For this review, take the finished solid that the model builds, in its own axes (mm). A direction names the side the tool comes from. Round coordinates to 2 decimals unless told otherwise and drop trailing zeros. Order: outer loops, then holes, each group sorted by start corner. A loop starts at its lowest first (then second) coordinate and runs counter-clockwise, first axis right, second up. Notation, with made-up numbers: M 5,33.25 L 9,33.25 A18 ccw 9,53.25 Z; hole C 11.25,60.25 d11. An arc over 180 degrees is marked long. Use a Markdown table: item, result.
from build123d import *

# Parameters (mm, degrees)
SKETCH1_W                              = 65
SKETCH1_H                              = 45
BOSS_EXTRUDE1_DEPTH                    = 45
SKETCH2_W                              = 15
SKETCH2_H                              = 10
CUT_EXTRUDE1_DEPTH                     = 40
SKETCH3_R                              = 5
BOSS_EXTRUDE2_DEPTH                    = 40
BOSS_EXTRUDE3_START                    = -40
BOSS_EXTRUDE3_DEPTH                    = 40
SKETCH5_R                              = 15
BOSS_EXTRUDE4_DEPTH                    = 2
CBORE_FOR_M2_HEX_CAP_SCREW2_AT_2_COUNT = 2
CBORE_FOR_M2_HEX_CAP_SCREW2_AT_2_PITCH = 50
CBORE_FOR_M2_HEX_CAP_SCREW2_AT_3_COUNT = 2
CBORE_FOR_M2_HEX_CAP_SCREW2_AT_3_PITCH = 35
CBORE_FOR_M2_HEX_CAP_SCREW2_AT_4_COUNT = 2
CBORE_FOR_M2_HEX_CAP_SCREW2_AT_4_PITCH = 61.032778079


with BuildPart() as part:
    # Sketch1 → Boss-Extrude1 (new body)
    with BuildSketch(Plane(origin=(0, 0, 0), x_dir=(1, 0, 0), z_dir=(0, 1, 0))):
        Rectangle(SKETCH1_W, SKETCH1_H)
    extrude(amount=BOSS_EXTRUDE1_DEPTH)

    # Sketch2 → Cut-Extrude1 (cut)
    with BuildSketch(Plane(origin=(0, 45, 0), x_dir=(1, 0, 0), z_dir=(0, 1, 0))):
        with Locations((-25, 17.5)):
            Rectangle(SKETCH2_W, SKETCH2_H)
        with Locations((-25, -17.5)):
            Rectangle(SKETCH2_W, SKETCH2_H)
        with Locations((25, -17.5)):
            Rectangle(SKETCH2_W, SKETCH2_H)
        with Locations((25, 17.5)):
            Rectangle(SKETCH2_W, SKETCH2_H)
    extrude(amount=-CUT_EXTRUDE1_DEPTH, mode=Mode.SUBTRACT)

    # Sketch3 → Boss-Extrude2 (add)
    with BuildSketch(Plane.XZ):
        with Locations(Location((0, 0, 0), (0, 0, 270))):
            Circle(SKETCH3_R)
    extrude(amount=BOSS_EXTRUDE2_DEPTH)

    # Sketch4 → Boss-Extrude3 (add)
    with BuildSketch(Plane.XZ.offset(40).offset(BOSS_EXTRUDE3_START)):
        with BuildLine():
            ThreePointArc((1.5, -4.769696007), (0.758788496, -4.942088629), (0, -5))
            ThreePointArc((0, -5), (-0.758788496, -4.942088629), (-1.5, -4.769696007))
            Line((-1.5, -4.769696007), (-1.5, -6.5))
            Line((-1.5, -6.5), (1.5, -6.5))
            Line((1.5, -6.5), (1.5, -4.769696007))
        make_face()
    extrude(amount=BOSS_EXTRUDE3_DEPTH)

    # Sketch5 → Boss-Extrude4 (add)
    with BuildSketch(Plane.XZ):
        with Locations(Location((0, 0, 0), (0, 0, 270))):
            Circle(SKETCH5_R)
    extrude(amount=BOSS_EXTRUDE4_DEPTH)

    # Sketch8 → CBORE for M2 Hex Cap Screw1 (revolve, cut)
    with BuildSketch(Plane(origin=(0, -40, 0), x_dir=(0, 0, -1), z_dir=(1, 0, 0))):
        Polygon((0, 0), (0, 5.721032743), (1.2, 5), (1.2, 1.4), (3.8095, 1.4), (3.8095, 0.025), (3.8345, 0), align=None)
    revolve(axis=Axis((0, -46.35, 0), (0, 1, 0)), mode=Mode.SUBTRACT)

    # Sketch12 → CBORE for M2 Hex Cap Screw2 (revolve, cut)
    with BuildSketch(Plane(origin=(-25, 5, -17.5), x_dir=(0, 0, 1), z_dir=(1, 0, 0))):
        Polygon((0, 0), (0, 10.721032743), (1.2, 10), (1.2, 1.4), (3.8095, 1.4), (3.8095, 0.025), (3.8345, 0), align=None)
    cbore_for_m2_hex_cap_screw2 = revolve(axis=Axis((-25, 11.35, -17.5), (0, -1, 0)), mode=Mode.SUBTRACT)

    # CBORE for M2 Hex Cap Screw2 at 2: CBORE for M2 Hex Cap Screw2 ×2
    with Locations(*[(i * CBORE_FOR_M2_HEX_CAP_SCREW2_AT_2_PITCH, 0, 0) for i in range(1, CBORE_FOR_M2_HEX_CAP_SCREW2_AT_2_COUNT)]):
        add(cbore_for_m2_hex_cap_screw2, mode=Mode.SUBTRACT)

    # CBORE for M2 Hex Cap Screw2 at 3: CBORE for M2 Hex Cap Screw2 ×2
    with Locations(*[(0, 0, i * CBORE_FOR_M2_HEX_CAP_SCREW2_AT_3_PITCH) for i in range(1, CBORE_FOR_M2_HEX_CAP_SCREW2_AT_3_COUNT)]):
        add(cbore_for_m2_hex_cap_screw2, mode=Mode.SUBTRACT)

    # CBORE for M2 Hex Cap Screw2 at 4: CBORE for M2 Hex Cap Screw2 ×2
    with Locations(*[Vector(0.8192319205190405, 0, 0.5734623443633283) * (i * CBORE_FOR_M2_HEX_CAP_SCREW2_AT_4_PITCH) for i in range(1, CBORE_FOR_M2_HEX_CAP_SCREW2_AT_4_COUNT)]):
        add(cbore_for_m2_hex_cap_screw2, mode=Mode.SUBTRACT)


solid = part.part
Q1. Draft analysis for pull direction X (two halves, no side actions). For faces 5 (the flat face through (32.5, 22, 0)), 6 (the flat face through (-32.5, 22, 0)), 7 (the cylindrical face through (23.81, 1.83, 17.34)), 8 (the cylindrical face through (28.38, 4.3, 19.26)), state which applies: pulls with the +X half, pulls with the -X half, needs draft (parallel to the pull), parting line crosses it, or undercut.
Determined:
| item | result |
|---|---|
| face 5 | pulls with the +X half |
| face 6 | pulls with the -X half |
| face 7 | undercut |
| face 8 | undercut |
Q2. Machinability: for faces 1 (the cylindrical face through (0.66, -0.986, 14.985)), 2 (the cylindrical face through (23.856, 4.297, -13.866)), 3 (the flat face through (-17.5, 25, -17)), 4 (the flat face through (0, -21, -6.5)), which of the approach directions +Z, -Z, +X, -X, +Y, -Y give a long, thin tool a straight path to every point of the face, cutting with its end or side? Answer none if there is none.
Determined:
| item | result |
|---|---|
| face 1 | -Y |
| face 2 | +Y |
| face 3 | -Z, -X, +Y |
| face 4 | -Z, +X, -X, -Y |
Q3. Clearance check with flat-ended pins moving along their axes: pin 1 (8 mm diameter, centred on x = -7, y = -22, fed in from -Z); pin 2 (5 mm diameter, centred on x = 27, z = 15.5, fed in from +Y); pin 3 (3 mm diameter, centred on x = -7, z = -5.5, fed in from -Y); pin 4 (16.5 mm diameter, centred on x = -23, y = 34.5, fed in from -Z). State where each tip first meets the part, or that it passes through.
Determined:
| item | result |
|---|---|
| pin 1 | stops at z = -4 |
| pin 2 | stops at y = 5 |
| pin 3 | stops at y = -2 |
| pin 4 | stops at z = -22.5 |
Q4. Add section C-C (y = 39). Write out the cut boundary in (x, z).
Determined:
| item | result |
|---|---|
| outline | M -32.5,-12.5 L -17.5,-12.5 L -17.5,-22.5 L 17.5,-22.5 L 17.5,-12.5 L 32.5,-12.5 L 32.5,12.5 L 17.5,12.5 L 17.5,22.5 L -17.5,22.5 L -17.5,12.5 L -32.5,12.5 Z |
Q5. Add section A-A (x = -25). Give the number of separate pieces and of enclosed holes in the cut face, then the cut area to 3 significant figures.
Determined:
| item | result |
|---|---|
| separate pieces | 3 |
| enclosed holes | 0 |
| area | 1,190 mm^2 |
Q6. Add section D-D (x = 14). Write out the cut boundary in (y, z).
Determined:
| item | result |
|---|---|
| outline | M -2,-5.39 L 0,-5.39 L 0,-22.5 L 45,-22.5 L 45,22.5 L 0,22.5 L 0,5.39 L -2,5.39 Z |
Q7. Wall thickness on line 1 along X through (y, z) = (4.4, 17.5); line 2 along X through (y, z) = (-37, 0); line 3 along X through (y, z) = (-39.45, 0): over which ranges is each line inside the solid? List them lowest first. Write a range as [from, to].
Determined:
| item | result |
|---|---|
| line 1 | x = [-32.5, -28.81], [-21.19, 21.19], [28.81, 32.5] |
| line 2 | x = [-5, -1.2], [1.2, 5] |
| line 3 | x = [-5, -3.81], [3.81, 5] |
